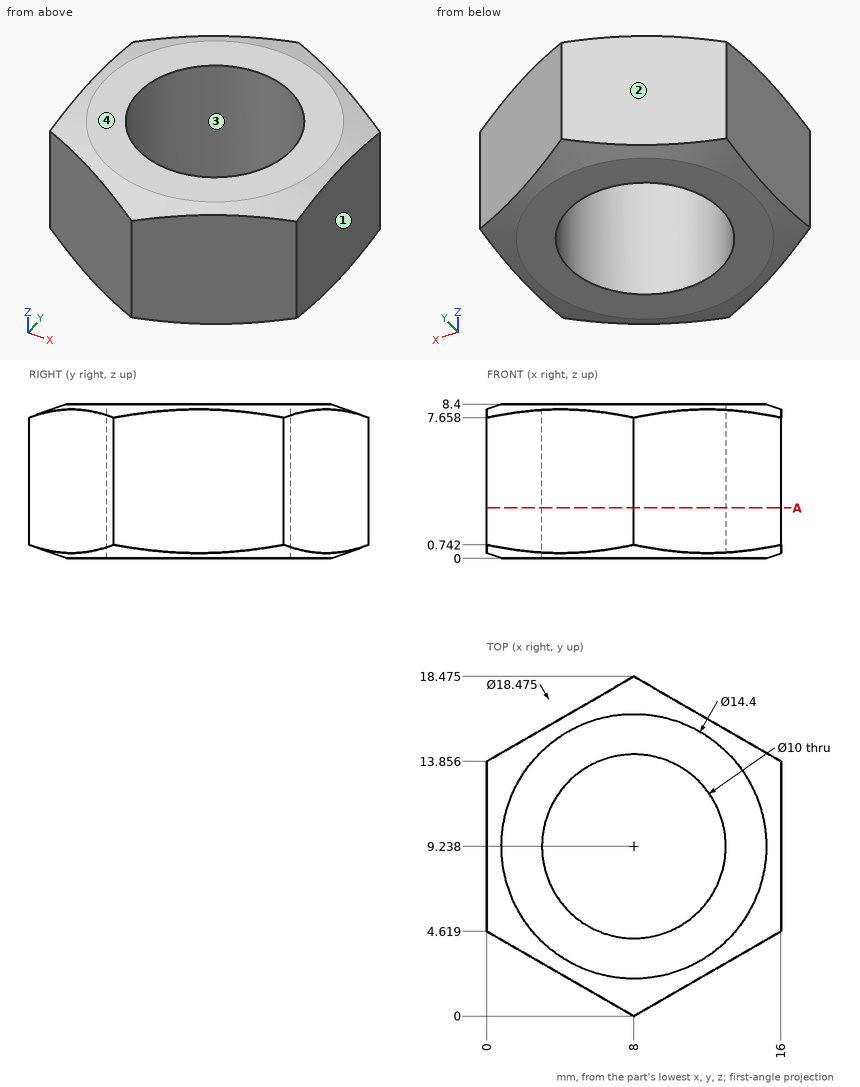
Input: dimensioned drawing with shaded views. Units: mm. Origin: part minimum x, y, z. Coordinates: 2 decimals unless noted, no trailing zeros. Loops run counter-clockwise (first coordinate to the right, second up) from the corner with the lowest first, then second, coordinate; pieces in that order, holes last. Notation, with made-up numbers: M -31,-37.5 L 14,-37.5 A19 cw 14,-27.5 Z; hole C -35,23.5 d8. An arc over 180 degrees is marked long. One line per item, written item: value. Start each with the question number.
1) Cut plane A-A (z = 2.75). Return loops of the section in (x, y) (1 decimal).
2) Material intervals for L1, parallel to Y at x = 5.75, z = 2.5 (1 decimal); L2, parallel to X at y = 7.25, z = 6; L3, parallel to Y at x = 4.75, z = 7.25 (1 decimal), sorted ascending. Write a range as from..to.
3) Pin query (flat end, axial travel): P1, Ø3, axis at y = 15, z = 4, coming from the -X side; P2, Ø1.5, axis at x = 7, z = 2.5, coming from the +Y side; P3, Ø2, axis at y = 15.5, z = 2, coming from the -X side (1 decimal). Return the tip coordinate at first contact, or that it passes through.
4) Draft query along X for the marked faces 1, 2, 3 and 4. Return one class per face: released by +X, released by -X, zero draft, split by the parting line, or undercut.
Evaluation:
1. outline: M 0,4.6 L 8,0 L 16,4.6 L 16,13.9 L 8,18.5 L 0,13.9 Z; hole C 8,9.2 d10
2. L1: 1.3..4.8, 13.7..17.2
2. L2: 0..3.41, 12.59..16
2. L3: 1.9..5.4, 13..16.6
3. P1: x = 0
3. P2: y = 18.33
3. P3: x = 1.1
4. face 1: released by +X
4. face 2: released by -X
4. face 3: undercut
4. face 4: zero draft
